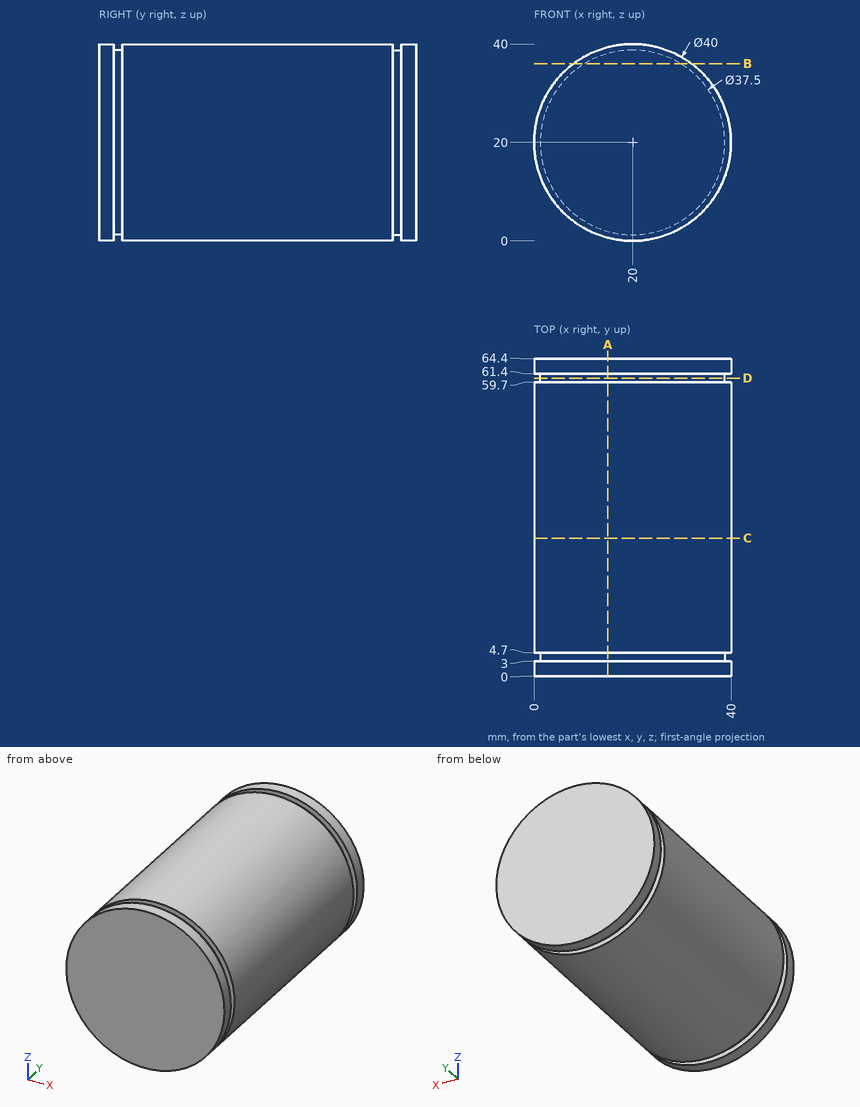
For this review, use the dimensioned drawing (mm, ordinates from the lowest corner) and the shaded views. Give positions to 0.01 mm unless a question says otherwise; leave off trailing zeros. Order: outer loops, then holes, each group sorted by start corner. A loop starts at its lowest first (then second) coordinate and runs counter-clockwise, first axis right, second up. Notation, with made-up numbers: M 40,63 L 64,63 A7 cw 64,72 Z; hole C 71.5,16 d2. An arc over 180 degrees is marked long. One line per question, with ' | ' between items. Start each with the question number.
1) Wall thickness on L1, parallel to Y at x = 8.5, z = 35.5; L2, parallel to X at y = 31, z = 13 (3 decimals); L3, parallel to Z at x = 16, y = 52.5: over which ranges is each line inside the solid? List them lowest first. Write a range as from..to.
2) Consider section C-C, the plane y = 28. Give the boundary of the cut face in (x, z).
3) Consider section D-D, the plane y = 60.5. Give the boundary of the cut face in (x, z), then the cut area to 3 significant figures.
4) Consider section A-A, the plane x = 15. Give the boundary of the cut face in (y, z).
5) Consider section B-B, the plane z = 36. Give the boundary of the cut face in (x, y), then the cut area to 3 significant figures.
6) Clearance check with flat-ended pins moving along their axes: P1, Ø10, axis at x = 33, z = 4.5, coming from the +Y side; P2, Ø4, axis at x = 25, y = 51.5, coming from the -Z side; P3, Ø2, axis at y = 7.5, z = 11.5, coming from the +X side; P4, Ø8, axis at y = 15, z = 12, coming from the +X side. State where each tip first meets the part, or that it passes through.
Found:
1) L1: y = 0..3, 4.7..59.7, 61.4..64.4 | L2: x = 1.265..38.735 | L3: z = 0.4..39.6
2) outline: C 20,20 d40
3) outline: C 20,20 d37.5 | area: 1,100 mm²
4) outline: M 0,0.64 L 3,0.64 L 3,1.93 L 4.7,1.93 L 4.7,0.64 L 59.7,0.64 L 59.7,1.93 L 61.4,1.93 L 61.4,0.64 L 64.4,0.64 L 64.4,39.36 L 61.4,39.36 L 61.4,38.07 L 59.7,38.07 L 59.7,39.36 L 4.7,39.36 L 4.7,38.07 L 3,38.07 L 3,39.36 L 0,39.36 Z
5) outline: M 8,0 L 32,0 L 32,3 L 29.78,3 L 29.78,4.7 L 32,4.7 L 32,59.7 L 29.78,59.7 L 29.78,61.4 L 32,61.4 L 32,64.4 L 8,64.4 L 8,61.4 L 10.22,61.4 L 10.22,59.7 L 8,59.7 L 8,4.7 L 10.22,4.7 L 10.22,3 L 8,3 Z | area: 1,530 mm²
6) P1: stops at y = 64.4 | P2: stops at z = 0.23 | P3: stops at x = 38.54 | P4: stops at x = 39.6
